```python
from build123d import *

# Parameters (mm, degrees)
SKETCH1_R               = 110
SKETCH1_R_2             = 8.75
BOSS_EXTRUDE1_DEPTH     = 26
CUT_EXTRUDE2_DEPTH      = 158.721273137
CUT_EXTRUDE2_DEPTH_BACK = 158.721273137
SKETCH3_R               = 58


with BuildPart() as part:
    # Sketch1 → Boss-Extrude1 (new body)
    with BuildSketch(Plane.XY):
        with Locations(Location((0, 0, 0), (0, 0, 180))):
            Circle(SKETCH1_R)
        with Locations(Location((0, 90, 0), (0, 0, 180))):
            Circle(SKETCH1_R_2, mode=Mode.SUBTRACT)
        with Locations(Location((63.639610307, 63.639610307, 0), (0, 0, 180))):
            Circle(SKETCH1_R_2, mode=Mode.SUBTRACT)
        with Locations(Location((90, 0, 0), (0, 0, 180))):
            Circle(SKETCH1_R_2, mode=Mode.SUBTRACT)
        with Locations(Location((63.639610307, -63.639610307, 0), (0, 0, 180))):
            Circle(SKETCH1_R_2, mode=Mode.SUBTRACT)
        with Locations(Location((0, -90, 0), (0, 0, 180))):
            Circle(SKETCH1_R_2, mode=Mode.SUBTRACT)
        with Locations(Location((-63.639610307, -63.639610307, 0), (0, 0, 180))):
            Circle(SKETCH1_R_2, mode=Mode.SUBTRACT)
        with Locations(Location((-90, 0, 0), (0, 0, 180))):
            Circle(SKETCH1_R_2, mode=Mode.SUBTRACT)
        with Locations(Location((-63.639610307, 63.639610307, 0), (0, 0, 180))):
            Circle(SKETCH1_R_2, mode=Mode.SUBTRACT)
    extrude(amount=BOSS_EXTRUDE1_DEPTH)

    # Sketch3 → Cut-Extrude2 (cut, two sides: drawn at the far end of the back side and taken through both)
    with BuildSketch(Plane.XY.offset(26).offset(-CUT_EXTRUDE2_DEPTH_BACK)):
        Circle(SKETCH3_R)
    extrude(amount=CUT_EXTRUDE2_DEPTH + CUT_EXTRUDE2_DEPTH_BACK, mode=Mode.SUBTRACT)

    # Sketch4 → Cut-Revolve1 (revolve, cut)
    with BuildSketch(Plane(origin=(0, 0, 0), x_dir=(1, 0, 0), z_dir=(0, 1, 0)), mode=Mode.PRIVATE) as cut_revolve1_sk:
        Polygon((79, 0), (81, -3), (110, -3), (110, 0), align=None)
    revolve(cut_revolve1_sk.sketch.rotate(Axis((0, 0, 0), (0, 0, 1)), 180), axis=Axis((0, 0, 0), (0, 0, 1)), mode=Mode.SUBTRACT)


solid = part.part
```
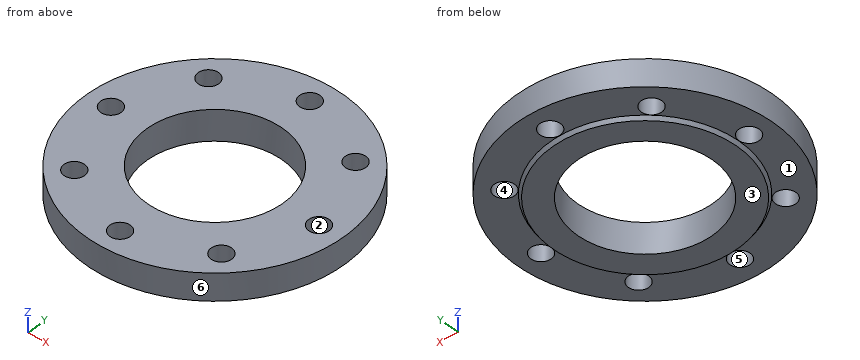
Build history of the part. All positions in model axes, mm. Face numbers are marked on the shaded views. A direction names the side the tool comes from. Round coordinates to 2 decimals unless told otherwise and drop trailing zeros. Loops run counter-clockwise (first coordinate to the right, second up) from the corner with the lowest first, then second, coordinate; pieces in that order, holes last.
Item 1: Which spindle directions (+Z, -Z, +X, -X, +Y, -Y) get a long thin tool onto all of the face, cutting with end or side? Do the marked faces 1 and 2. Say none if no direction does.
Item 2: Pin check, flat tips, straight feed: P1, Ø12, axis at x = -26, z = 6, coming from the +Y side; P2, Ø2, axis at x = -25, z = 11, coming from the -Y side; P3, Ø12, axis at x = -54, y = 82, coming from the -Z side. Stop position of each tip, or through.
Item 3: Drill centre lines: line 1 along X through (y, z) = (1, 17.25); line 2 along Y through (x, z) = (0, 15.75); line 3 along Y through (x, z) = (1.5, 14). Where is each one in solid material? Low to high.
Item 4: Saw through at A-A (x = 0). List the corners of the cut face in (y, z).
Item 5: Two-plate mould, pull along Y, no slides. Class the marked faces 3, 4, 5 and 6: released by +Y, released by -Y, zero draft, split by the parting line, or undercut.
Item 6: Saw through at D-D (x = 90). List the corners of the cut face in (y, z), then the cut area to 3 significant figures.
Item 7: Saw through at C-C (z = 17.75). State how many separate pieces and enclosed holes the cut face has, then the cut area to 3 significant figures.
Worked answers:
1. face 1: -Z
1. face 2: +Z, -Z
2. P1: stops at y = 108.17
2. P2: stops at y = -107.35
2. P3: stops at z = 3
3. line 1: x = -110 to -98.69, -81.31 to -57.99, 57.99 to 81.31, 98.69 to 110
3. line 2: y = -110 to -98.75, -81.25 to -58, 58 to 81.25, 98.75 to 110
3. line 3: y = -109.99 to -98.62, -81.38 to -57.98, 57.98 to 81.38, 98.62 to 109.99
4. outline: (-110, 3) - (-98.75, 3) - (-98.75, 26) - (-110, 26) - close; (-81.25, 3) - (-81, 3) - (-79, 0) - (-58, 0) - (-58, 26) - (-81.25, 26) - close; (58, 0) - (79, 0) - (81, 3) - (81.25, 3) - (81.25, 26) - (58, 26) - close; (98.75, 3) - (110, 3) - (110, 26) - (98.75, 26) - close
5. face 3: zero draft
5. face 4: undercut
5. face 5: undercut
5. face 6: split by the parting line
6. outline: (-63.25, 3) - (-8.75, 3) - (-8.75, 26) - (-63.25, 26) - close; (8.75, 3) - (63.25, 3) - (63.25, 26) - (8.75, 26) - close
6. area: 2,510 mm2
7. separate pieces: 1
7. enclosed holes: 9
7. area: 25,500 mm2
